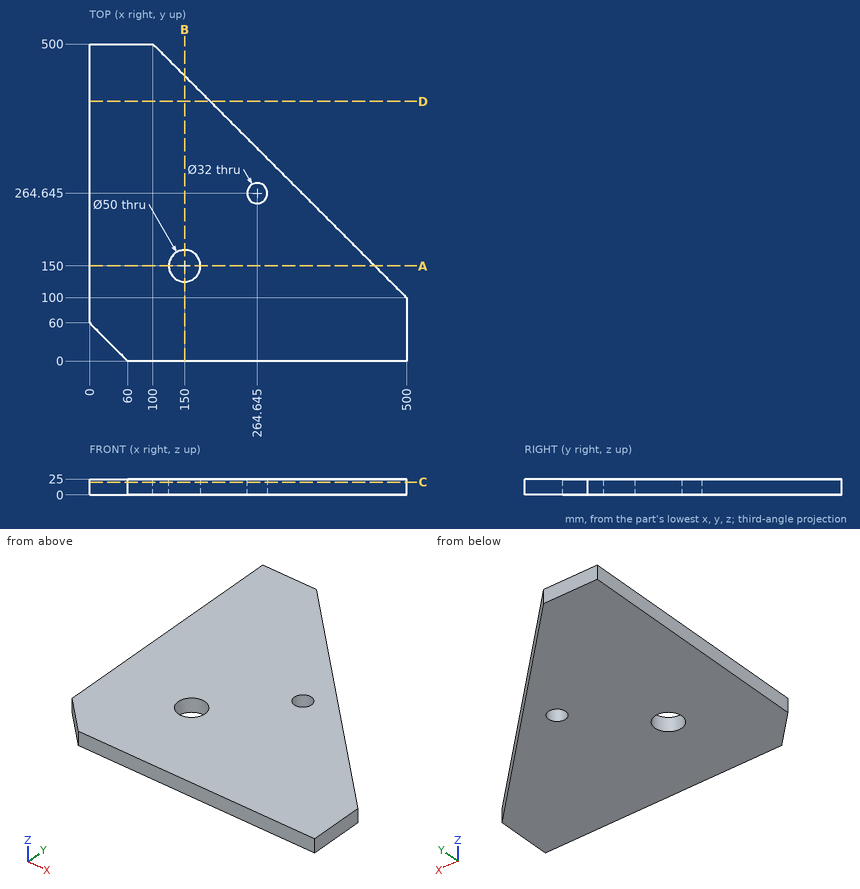
Design review of the part shown in the three views and the two pictorial views. Dimensions are in mm from the part's minimum x, y and z. Round coordinates to 2 decimals unless told otherwise and drop trailing zeros. Write each loop counter-clockwise with the first axis right and the second up, starting at its lowest first coordinate (ties: lowest second). Pieces come first, ordered by that corner, then holes.
Item 1: Consider section A-A on y = 150. Give the boundary of the cut face in (x, z), and give its area (3 significant figures).
Item 2: Consider section D-D on y = 409.5. Give the boundary of the cut face in (x, z), and give its area (3 significant figures).
Item 3: Wall thickness on L1, parallel to X at y = 264.5, z = 15.5 (1 decimal); L2, parallel to Y at x = 150, z = 14; L3, parallel to X at y = 167, z = 11.75: over which ranges is each line inside the solid? List them lowest first.
Item 4: For pin 1 Ø1 at (x, z) = (269, 10.5) entering from +Y; pin 2 Ø5 at (y, z) = (346.5, 7) entering from +X; pin 3 Ø5 at (y, z) = (406, 7.5) entering from +X, all flat-tipped, find the tip position at first contact; note any pin that passes through.
Item 5: Consider section C-C on z = 20. Give the boundary of the cut face in (x, y) (1 decimal), and give its area (3 significant figures).
Check values:
1. outline: (0, 0) - (125, 0) - (125, 25) - (0, 25) - close; (175, 0) - (450, 0) - (450, 25) - (175, 25) - close
1. area: 10,000 mm2
2. outline: (0, 0) - (190.5, 0) - (190.5, 25) - (0, 25) - close
2. area: 4,760 mm2
3. L1: x = 0 to 248.6, 280.6 to 335.5
3. L2: y = 0 to 125, 175 to 450
3. L3: x = 0 to 131.67, 168.33 to 433
4. pin 1: stops at y = 331.5
4. pin 2: stops at x = 256
4. pin 3: stops at x = 196.5
5. outline: (0, 60) - (60, 0) - (500, 0) - (500, 100) - (100, 500) - (0, 500) - close; hole circle Ø50 at (150, 150); hole circle Ø32 at (264.6, 264.6)
5. area: 165,000 mm2
